```python
from build123d import *

# Parameters (mm, degrees)
SKETCH2_R = 2


with BuildPart() as part:
    # Sweep1: sweep along a curve in space
    with BuildLine() as sweep1_path:
        Line((-19.39826571, 55.978701071, 2.254926967), (-16.715694993, 55.978701071, 2.254926967))
        ThreePointArc((-6.047634181, 59.123559398, -3.439623567), (-10.468184265, 56.826927396, 0.719001604), (-16.715694993, 55.978701071, 2.254926967))
        Line((-6.047634181, 59.123559398, -3.439623567), (-4.269895959, 60.792120921, -6.460970453))
        ThreePointArc((0.98288182, 55.507835041, -21.708417726), (-0.455385422, 61.380619924, -14.795022607), (-4.269895959, 60.792120921, -6.460970453))
        Line((0.98288182, 55.507835041, -21.708417726), (0.488315483, 34.167885645, -33.784564331))
        ThreePointArc((12.48587526, 23.513552475, -39.813786189), (3.915464358, 26.647289087, -38.040423843), (0.488315483, 34.167885645, -33.784564331))
        Line((12.48587526, 23.513552475, -39.813786189), (39.17173429, 23.513552475, -39.813786189))
    # Sketch2 → Sweep1 (sweep)
    with BuildSketch(Plane(origin=(-19.39826571, 0, 0), x_dir=(0, 0, -1), z_dir=(1, 0, 0))):
        with Locations((-2.254926967, 55.978701071)):
            Circle(SKETCH2_R)
    sweep(path=sweep1_path.line)


solid = part.part
```
Geometry check sheet. Reference: the model listing, model coordinates, mm. A direction names the side the tool comes from. Give positions to 0.01 mm unless a question says otherwise; leave off trailing zeros. Loops run counter-clockwise (first coordinate to the right, second up) from the corner with the lowest first, then second, coordinate; pieces in that order, holes last. Notation, with made-up numbers: M 16.25,66.5 L 27.25,66.5 A25 cw 27.25,96.5 Z; hole C -27.5,24 d8. An arc over 180 degrees is marked long. Write item = value, one per line. Start each with the question number.
1. Section check A-A, the plane x = 26. Enter the section's corners in (y, z).
2. Thickness scan on probe 1 along Z at (x, y) = (-1, 33.5); probe 2 along X at (y, z) = (61, -17); probe 3 along Z at (x, y) = (1.5, 35). Record the ranges inside material, lowest first.
3. Tool access check on faces 1 (the face through (26.016, 22.076, -41.204)), 2 (the face through (-18.04, 57.96, 2.52)), 3 (the face through (39.172, 23, -40)). Record the directions out of +Z, -Z, +X, -X, +Y, -Y that give a thin tool (end or side, any length) a straight path to the whole face; none if there is none.
4. Go/stop test with flat-tipped pins: P1, Ø8, axis at y = 47, z = -25.5, coming from the -X side; P2, Ø10, axis at x = 5.5, y = 38, coming from the +Z side; P3, Ø12, axis at y = 41, z = -31, coming from the -X side. Record where each tip stops, or that it passes through.
Values follow:
q1.outline = C 23.51,-39.81 d4
q2.probe_1 = -35.62 to -32.63
q2.probe_2 = -1.82 to 2.13
q2.probe_3 = -35.3 to -31.31
q3.face_1 = +X
q3.face_2 = -X
q3.face_3 = +Z, -Z, +X, +Y, -Y
q4.P1 = -1.28
q4.P2 = -27.81
q4.P3 = -1.48
